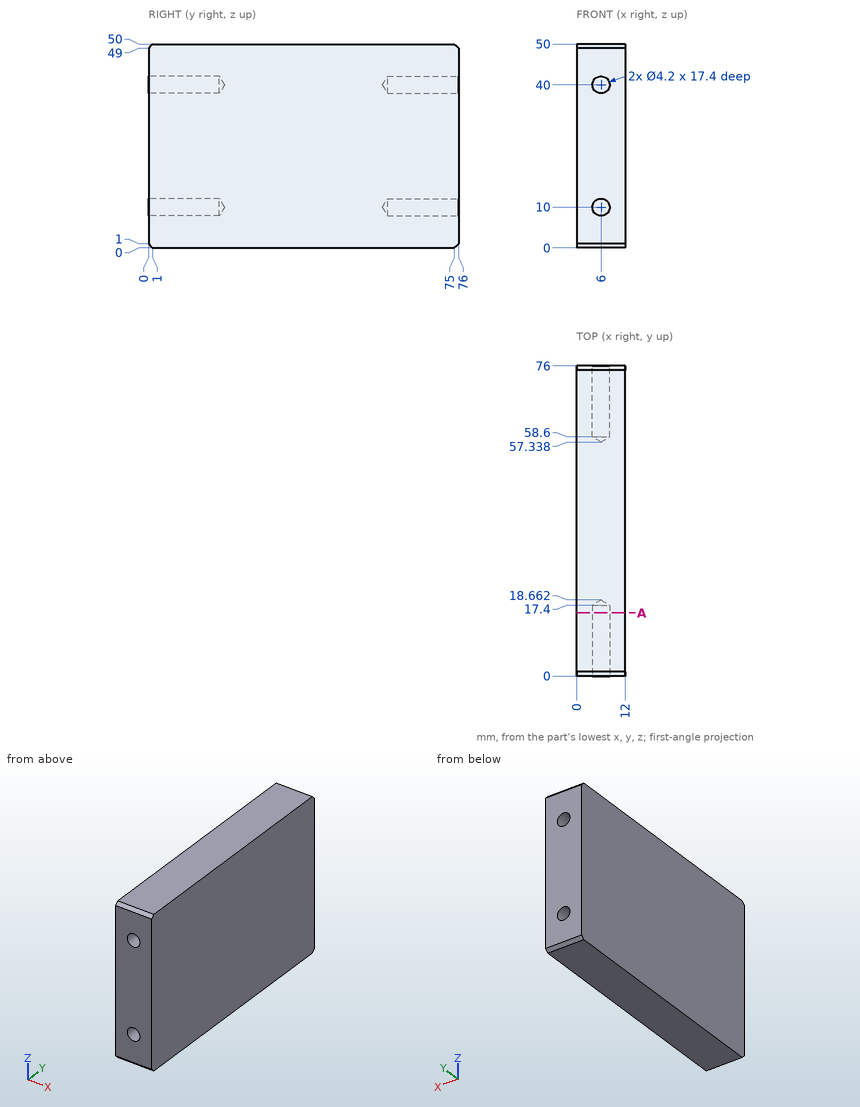
Geometry check sheet. Reference: drawing and pictorial views, mm from the part's lowest x, y, z. Give positions to 0.01 mm unless a question says otherwise; leave off trailing zeros. Loops run counter-clockwise (first coordinate to the right, second up) from the corner with the lowest first, then second, coordinate; pieces in that order, holes last. Notation, with made-up numbers: (17, 68) - (39, 68) arc R15 ccw to (39, 75) - close; hole circle Ø10 at (50.25, 22.5). An arc over 180 degrees is marked (long way). One line per question, with ' | ' between items. Start each with the question number.
1. Cross-section at A-A, the plane y = 15.5. Enter the section's corners in (x, z), plus the area to 3 significant figures.
2. Material ranges on line 1 along Z through (x, y) = (6.25, 16) (1 decimal); line 2 along X through (y, z) = (10, 10); line 3 along Z through (x, y) = (4.25, 68), recorded low to high. Write a range as [from, to].
3. Gauge pin test, flat end, axial feed: pin 1 Ø5.5 at (x, z) = (6, 40) entering from +Y. Record the tip position at first contact, or that the pin passes through.
Check result:
1) outline: (0, 0) - (12, 0) - (12, 50) - (0, 50) - close; hole circle Ø4.2 at (6, 10); hole circle Ø4.2 at (6, 40) | area: 572 mm2
2) line 1: z = [0, 7.9], [12.1, 37.9], [42.1, 50] | line 2: x = [0, 3.9], [8.1, 12] | line 3: z = [0, 8.84], [11.16, 38.84], [41.16, 50]
3) pin 1: stops at y = 76
